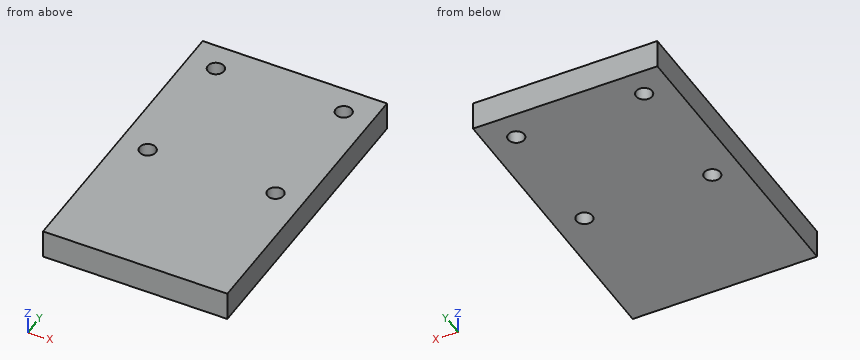
from build123d import *

# Parameters (mm, degrees)
SKETCH_1_W          = 160
SKETCH_1_H          = 260
EXTRUDE_1_DEPTH     = 25
HOLE_WIZARD_M16_1_D = 14


with BuildPart() as part:
    # 草图1 → 凸台-拉伸1 (new body)
    with BuildSketch(Plane.XY):
        Rectangle(SKETCH_1_W, SKETCH_1_H)
    extrude(amount=EXTRUDE_1_DEPTH)

    # M16 螺纹孔1 (through all)
    with Locations(Plane.XY.offset(25)):
        with Locations((-55.5, 105.5), (-55.5, -5.5), (55.5, -5.5), (55.5, 105.5)):
            Hole(HOLE_WIZARD_M16_1_D / 2)


solid = part.part
Verification items for the finished model (mm, model axes). Give positions to 0.01 mm unless a question says otherwise; leave off trailing zeros. Write each loop counter-clockwise with the first axis right and the second up, starting at its lowest first coordinate (ties: lowest second). Pieces come first, ordered by that corner, then holes. Notation, with made-up numbers: (28, -15.75) -> (72, -15.75) arc R35 ccw to (72, 17.25) -> close; hole circle Ø11 at (49.25, 4). An arc over 180 degrees is marked (long way). Use CSV: the item, a comma, the result in double quotes.
(1) Sectioned sample at B-B (x = -55.5). Record the cut outline in (y, z).
Derived:
outline,"(-130, 0) -> (-12.5, 0) -> (-12.5, 25) -> (-130, 25) -> close; (1.5, 0) -> (98.5, 0) -> (98.5, 25) -> (1.5, 25) -> close; (112.5, 0) -> (130, 0) -> (130, 25) -> (112.5, 25) -> close"
(2) Material ranges on L1, parallel to Y at x = -55.5, z = 8.5; L2, parallel to Y at x = -56.5, z = 3, recorded low to high.
Derived:
L1,"y = -130 to -12.5, 1.5 to 98.5, 112.5 to 130"
L2,"y = -130 to -12.43, 1.43 to 98.57, 112.43 to 130"
(3) Sectioned sample at A-A (y = -5.5). Record the cut outline in (x, z), plus the area to 3 significant figures.
Derived:
outline,"(-80, 0) -> (-62.5, 0) -> (-62.5, 25) -> (-80, 25) -> close; (-48.5, 0) -> (48.5, 0) -> (48.5, 25) -> (-48.5, 25) -> close; (62.5, 0) -> (80, 0) -> (80, 25) -> (62.5, 25) -> close"
area,"3,300 mm^2"
